Can you work these out from the drawing? Everything is in mm from the part's minimum corner. Round coordinates to 2 decimals unless told otherwise and drop trailing zeros. Order: outer loops, then holes, each group sorted by start corner. A loop starts at its lowest first (then second) coordinate and runs counter-clockwise, first axis right, second up. Notation, with made-up numbers: (-33, 76) - (-19, 76) arc R23 ccw to (-19, 112) - close; hole circle Ø3 at (-8, 49.5). An arc over 180 degrees is marked (long way). Answer as a JSON object with one key per item and string values.
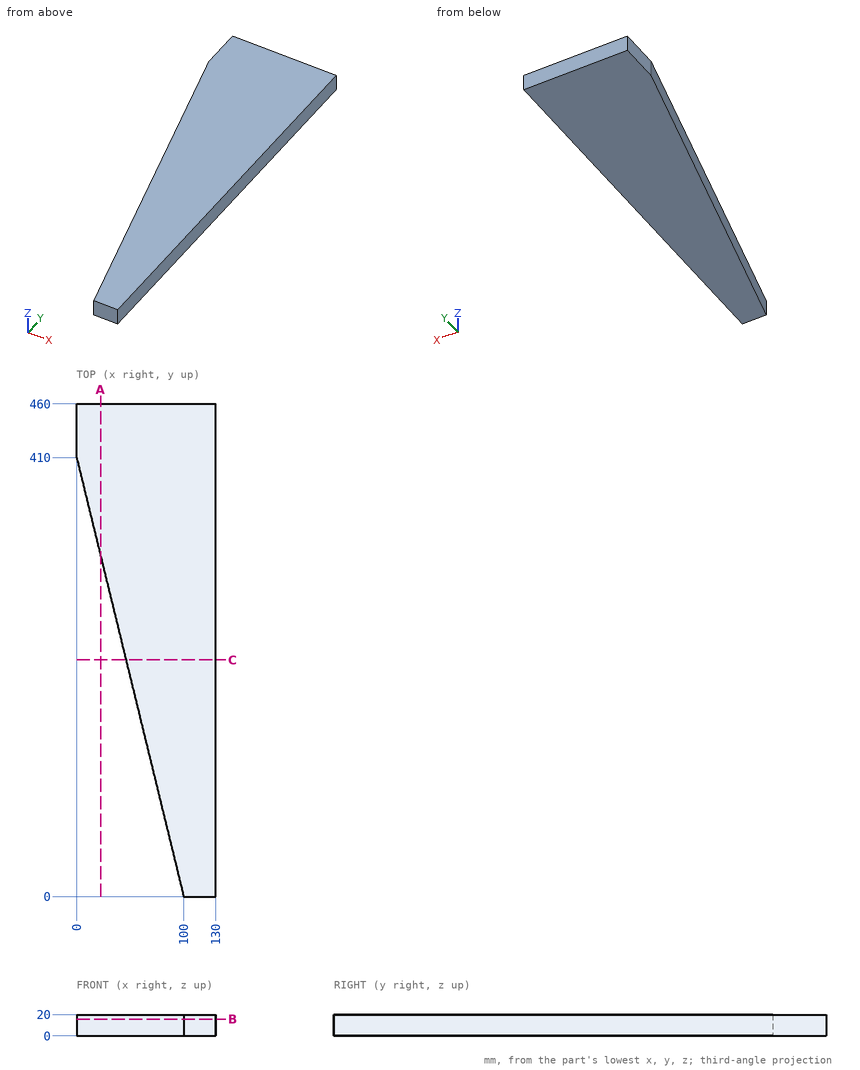
1. Imagine slicing it at A-A (x = 22.5). List the corners of the cut face in (y, z) for me.
Responses:
{"outline": "(317.75, 0) - (460, 0) - (460, 20) - (317.75, 20) - close"}
2. Imagine slicing it at C-C (y = 221). List the corners of the cut face in (x, z) for me.
Responses:
{"outline": "(46.1, 0) - (130, 0) - (130, 20) - (46.1, 20) - close"}
3. Imagine slicing it at B-B (z = 15.75). List the corners of the cut face in (x, y) for me.
Responses:
{"outline": "(0, 410) - (100, 0) - (130, 0) - (130, 460) - (0, 460) - close"}
4. For P1, Ø2, axis at y = 270, z = 13.5, coming from the -X side; P2, Ø5, axis at y = 396, z = 11.5, coming from the -X side, each with a flat end and sliding along its axis, tell me the tip position at first contact or that it passes through.
Responses:
{"P1": "x = 33.9", "P2": "x = 2.8"}
5. If I drill on L1, parallel to X at y = 191, z = 6.5; L2, parallel to X at y = 216.5, z = 4.75, over which ranges is the centre line in solid material (lowest first)? Write a range as [from, to].
Responses:
{"L1": "[53.41, 130]", "L2": "[47.2, 130]"}
